The listing builds one solid part. Answer for the finished solid, in the listing's coordinates (mm). A direction names the side the tool comes from. Give positions to 0.01 mm unless a question says otherwise; leave off trailing zeros. Order: outer loops, then holes, each group sorted by start corner. A loop starts at its lowest first (then second) coordinate and runs counter-clockwise, first axis right, second up. Notation, with made-up numbers: M 37,11.5 L 60,11.5 A14 ccw 60,27.5 Z; hole C 76.5,77.25 d8. An arc over 180 degrees is marked long. Answer as a JSON object with one key per item and string values. Group by question number.
```python
from build123d import *

# Parameters (mm, degrees)
SKETCH1_W             = 54
SKETCH1_H             = 70
BOSS_EXTRUDE1_DEPTH   = 48
SKETCH2_W             = 106
SKETCH2_H             = 90
BOSS_EXTRUDE2_DEPTH   = 16
SKETCH3_W             = 78
SKETCH3_H             = 78
BOSS_EXTRUDE3_DEPTH   = 15
CHAMFER1_SIZE         = 5
SKETCH4_R             = 35.15
SKETCH4_R_2           = 31.35
CUT_EXTRUDE1_DEPTH    = 1.97
HOLE1_D               = 16
HOLE2_D               = 22
HOLE2_DEPTH           = 63
CHAMFER2_SIZE         = 1
M5_TAPPED_HOLE1_D     = 4.2
M5_TAPPED_HOLE1_DEPTH = 10
M5_TAPPED_HOLE1_TIP   = 1.2618073
HOLE3_D               = 6.4
HOLE3_CBORE_D         = 11
HOLE3_CBORE_DEPTH     = 9
SKETCH16_R            = 10.3
CUT_EXTRUDE2_DEPTH    = 3.8


with BuildPart() as part:
    # Sketch1 → Boss-Extrude1 (new body)
    with BuildSketch(Plane.XY):
        Rectangle(SKETCH1_W, SKETCH1_H)
    extrude(amount=BOSS_EXTRUDE1_DEPTH)

    # Sketch2 → Boss-Extrude2 (add)
    with BuildSketch(Plane.XY.offset(48)):
        Rectangle(SKETCH2_W, SKETCH2_H)
    extrude(amount=BOSS_EXTRUDE2_DEPTH)

    # Sketch3 → Boss-Extrude3 (add)
    with BuildSketch(Plane.XY.offset(64)):
        Rectangle(SKETCH3_W, SKETCH3_H)
    extrude(amount=BOSS_EXTRUDE3_DEPTH)

    # Chamfer1
    chamfer1_edges = [part.edges().sort_by_distance(p)[0] for p in [
        (-53, 45, 56),
        (-53, -45, 56),
        (53, -45, 56),
        (53, 45, 56),
        (-39, 39, 71.5),
        (-39, -39, 71.5),
        (39, -39, 71.5),
        (39, 39, 71.5),
        (27, -35, 24),
        (-27, -35, 24),
        (-27, 35, 24),
        (27, 35, 24),
    ]]
    chamfer(chamfer1_edges, length=CHAMFER1_SIZE)

    # Sketch4 → Cut-Extrude1 (cut)
    with BuildSketch(Plane.XY.offset(79)):
        Circle(SKETCH4_R)
        Circle(SKETCH4_R_2, mode=Mode.SUBTRACT)
    extrude(amount=-CUT_EXTRUDE1_DEPTH, mode=Mode.SUBTRACT)

    # Hole1 (through all)
    with Locations(Plane.XY.offset(79)):
        with Locations((0, -19), (0, 19)):
            Hole(HOLE1_D / 2)

    # Hole2
    with Locations(Plane(origin=(0, 0, 0), x_dir=(-1, 0, 0), z_dir=(0, 0, -1))):
        with Locations((0, 19), (0, -19)):
            Hole(HOLE2_D / 2, depth=HOLE2_DEPTH)

    # Chamfer2
    chamfer2_edges = [part.edges().sort_by_distance(p)[0] for p in [
        (8, 19, 79),
        (8, -19, 79),
        (-11, -19, 0),
        (-11, 19, 0),
    ]]
    chamfer(chamfer2_edges, length=CHAMFER2_SIZE)

    # M5 Tapped Hole1
    with Locations(Plane(origin=(0, 0, 0), x_dir=(-1, 0, 0), z_dir=(0, 0, -1))):
        with Locations((20, -19), (20, 19), (-20, 19), (-20, -19)):
            Hole(M5_TAPPED_HOLE1_D / 2, depth=M5_TAPPED_HOLE1_DEPTH)
            with Locations((0, 0, -(M5_TAPPED_HOLE1_DEPTH + M5_TAPPED_HOLE1_TIP / 2))):  # 118° drill point
                Cone(0, M5_TAPPED_HOLE1_D / 2, M5_TAPPED_HOLE1_TIP, mode=Mode.SUBTRACT)

    # Hole3 (through all)
    with Locations(Plane(origin=(0, 0, 48), x_dir=(-1, 0, 0), z_dir=(0, 0, -1))):
        with Locations((45, -30), (45, 30), (-45, 30), (-45, -30)):
            CounterBoreHole(HOLE3_D / 2, HOLE3_CBORE_D / 2, HOLE3_CBORE_DEPTH)

    # Sketch16 → Cut-Extrude2 (cut)
    with BuildSketch(Plane.XY.offset(74)):
        with Locations((0, 19)):
            Circle(SKETCH16_R)
        with Locations((0, -19)):
            Circle(SKETCH16_R)
    extrude(amount=-CUT_EXTRUDE2_DEPTH, mode=Mode.SUBTRACT)


solid = part.part
```
Item 1: Section D-D (x = 15.5) is taken. Determine the outline of the cut face in (y, z), and give its area (3 significant figures).
Item 2: Consider probe 1 along Y at (x, z) = (45, 51.5); probe 2 along Y at (x, z) = (-45, 60); probe 3 along Y at (x, z) = (0, 78). Determine where each line is inside the solid, lowest interval first. Write a range as from..to.
Item 3: Section A-A (x = 45) is taken. Determine the outline of the cut face in (y, z).
Item 4: Determine the mould class of faces 4 (the flat face through (-36, 1, 48)), 5 (the flat face through (-37, 36, 71)), 6 (the flat face through (53, -1, 56)), 7 (the cylindrical face through (-41.948, 30.961, 60.549)) for opening direction X: released by +X, released by -X, zero draft, split by the parting line, or undercut.
Item 5: A tool of negligible diameter and unlimited length cuts with its end or side. For faces 1 (the flat face through (25, -32, 24)), 2 (the flat face through (-2, 11, 63)), 3 (the flat face through (27, 0, 24)), from which of +Z, -Z, +X, -X, +Y, -Y can it reach the whole face along a straight path? Write none if from no direction.
Item 6: Section C-C (y = 0) is taken. Determine the outline of the cut face in (x, z).
Item 7: Flat-ended cylindrical pins translate along their axes: P1, Ø2, axis at x = -7, y = 23, coming from the +Z side; P2, Ø7.5, axis at x = 2.5, z = 68, coming from the -Y side; P3, Ø2, axis at y = -22, z = 36, coming from the +X side; P4, Ø11, axis at x = -2.5, y = -20, coming from the -Z side. Find the tip coordinate at first contact, or state that the pin passes through.
Item 8: Section B-B (z = 25) is taken. Determine the outline of the cut face in (x, y).
Values found:
{
 "1": {"outline": "M -45,48 L -35,48 L -35,0 L 35,0 L 35,48 L 45,48 L 45,64 L 39,64 L 39,79 L 31.55,79 L 31.55,77.03 L 27.25,77.03 L 27.25,79 L -27.25,79 L -27.25,77.03 L -31.55,77.03 L -31.55,79 L -39,79 L -39,64 L -45,64 Z", "area": "5,950 mm^2"},
 "2": {"probe 1": "y = -45..-35.5, -24.5..24.5, 35.5..45", "probe 2": "y = -45..-33.2, -26.8..26.8, 33.2..45", "probe 3": "y = -39..-35.15, -31.35..-27, -11..11, 27..31.35, 35.15..39"},
 "3": {"outline": "M -45,48 L -35.5,48 L -35.5,57 L -33.2,57 L -33.2,64 L -45,64 Z; M -26.8,57 L -24.5,57 L -24.5,48 L 24.5,48 L 24.5,57 L 26.8,57 L 26.8,64 L -26.8,64 Z; M 33.2,57 L 35.5,57 L 35.5,48 L 45,48 L 45,64 L 33.2,64 Z"},
 "4": {"face 4": "zero draft", "face 5": "released by -X", "face 6": "released by +X", "face 7": "undercut"},
 "5": {"face 1": "-Z, +X, -Y", "face 2": "-Z", "face 3": "-Z, +X, +Y, -Y"},
 "6": {"outline": "M -53,48 L -27,48 L -27,0 L 27,0 L 27,48 L 53,48 L 53,64 L 39,64 L 39,79 L 35.15,79 L 35.15,77.03 L 31.35,77.03 L 31.35,79 L -31.35,79 L -31.35,77.03 L -35.15,77.03 L -35.15,79 L -39,79 L -39,64 L -53,64 Z"},
 "7": {"P1": "stops at z = 79", "P2": "stops at y = -39", "P3": "stops at x = 27", "P4": "stops at z = 63"},
 "8": {"outline": "M -27,-30 L -22,-35 L 22,-35 L 27,-30 L 27,30 L 22,35 L -22,35 L -27,30 Z; hole C 0,-19 d22; hole C 0,19 d22"}
}
